```python
from build123d import *

# Parameters (mm, degrees)
BOSS_EXTRUDE7_DEPTH  = 3
SKETCH7_R            = 3.674588618
BOSS_EXTRUDE8_DEPTH  = 3.5
SKETCH8_R            = 3.674588618
BOSS_EXTRUDE9_DEPTH  = 3.5
SKETCH9_R            = 3.674588618
BOSS_EXTRUDE10_DEPTH = 3
SKETCH10_R           = 3.674588618
BOSS_EXTRUDE11_DEPTH = 3
SKETCH11_R           = 4.731271099
BOSS_EXTRUDE12_DEPTH = 1
SKETCH12_R           = 3.75
BOSS_EXTRUDE13_DEPTH = 7
BOSS_EXTRUDE14_START = 1
SKETCH13_R           = 4.731271099
BOSS_EXTRUDE14_DEPTH = 1
BOSS_EXTRUDE15_START = 7
SKETCH14_R           = 3.75
BOSS_EXTRUDE15_DEPTH = 7
CHAMFER1_SIZE        = 0.5


with BuildPart() as part:
    # Sketch1 → Boss-Extrude7 (new body)
    with BuildSketch(Plane.XY):
        with BuildLine():
            Line((-7.464079644, 5.007711231), (7.464079644, 5.007711231))
            ThreePointArc((7.464079644, 5.007711231), (12.46407809, 0.007713678), (7.464080538, -4.992284768))
            Line((7.464080538, -4.992284768), (-7.464079644, -4.992286102))
            ThreePointArc((-7.464079644, -4.992286102), (-12.464078311, 0.007712565), (-7.464079644, 5.007711231))
        make_face()
    extrude(amount=-BOSS_EXTRUDE7_DEPTH)

    # Sketch7 → Boss-Extrude8 (add)
    with BuildSketch(Plane(origin=(0, 0, -3), x_dir=(-1, 0, 0), z_dir=(0, 0, -1))):
        with Locations(Location((7.464079644, 0.007712565, 0), (0, 0, 180))):
            Circle(SKETCH7_R)
    extrude(amount=BOSS_EXTRUDE8_DEPTH)

    # Sketch8 → Boss-Extrude9 (add)
    with BuildSketch(Plane.XY):
        with Locations((7.464079644, 0.007712565)):
            Circle(SKETCH8_R)
    extrude(amount=BOSS_EXTRUDE9_DEPTH)

    # Sketch9 → Boss-Extrude10 (add)
    # profile 1 of 2: a face of its own
    with BuildSketch(Plane(origin=(0, 0, -6.5), x_dir=(-1, 0, 0), z_dir=(0, 0, -1))):
        with BuildLine():
            Line((7.458914982, 5.007708564), (-0.003874001, 5.003854283))
            ThreePointArc((-0.003874001, 5.003854283), (-5.003216645, -0.001949753), (0.003880454, -4.999997327))
            Line((0.003880454, -4.999997327), (7.464079644, -4.992284768))
            ThreePointArc((7.464079644, -4.992284768), (12.464077644, 0.007713232), (7.464079644, 5.007711231))
            Line((7.464079644, 5.007711231), (7.458914982, 5.007708564))
        make_face()
        with Locations(Location((7.464079644, 0.007712565, 0), (0, 0, 180))):
            Circle(SKETCH9_R, mode=Mode.SUBTRACT)
    # profile 2 of 2: a face of its own
    with BuildSketch(Plane(origin=(0, 0, -6.5), x_dir=(-1, 0, 0), z_dir=(0, 0, -1))):
        with Locations(Location((7.464079644, 0.007712565, 0), (0, 0, 180))):
            Circle(SKETCH9_R)
    extrude(amount=BOSS_EXTRUDE10_DEPTH)

    # Sketch10 → Boss-Extrude11 (add)
    # profile 1 of 2: a face of its own
    with BuildSketch(Plane.XY.offset(3.5)):
        with BuildLine():
            ThreePointArc((-0.003873651, 5.003854283), (-5.003216178, -0.00216555), (0.004312288, -4.999996973))
            Line((0.004312288, -4.999996973), (7.3891908, -4.991725236))
            ThreePointArc((7.3891908, -4.991725236), (12.463938092, -0.029732908), (7.464079644, 5.007711231))
            Line((7.464079644, 5.007711231), (7.458914981, 5.007708564))
            Line((7.458914981, 5.007708564), (-0.003873651, 5.003854283))
        make_face()
        with Locations((7.464079644, 0.007712565)):
            Circle(SKETCH10_R, mode=Mode.SUBTRACT)
    # profile 2 of 2: a face of its own
    with BuildSketch(Plane.XY.offset(3.5)):
        with Locations((7.464079644, 0.007712565)):
            Circle(SKETCH10_R)
    extrude(amount=BOSS_EXTRUDE11_DEPTH)

    # Sketch11 → Boss-Extrude12 (add)
    with BuildSketch(Plane.XY.offset(6.5)):
        with Locations((1e-09, 0.015425152)):
            Circle(SKETCH11_R)
    extrude(amount=BOSS_EXTRUDE12_DEPTH)

    # Sketch12 → Boss-Extrude13 (add)
    with BuildSketch(Plane.XY.offset(7.5)):
        with Locations((1e-09, 0.015425152)):
            Circle(SKETCH12_R)
    extrude(amount=BOSS_EXTRUDE13_DEPTH)

    # Sketch13 → Boss-Extrude14 (add)
    with BuildSketch(Plane(origin=(0, 0, -9.5), x_dir=(-1, 0, 0), z_dir=(0, 0, -1)).offset(BOSS_EXTRUDE14_START)):
        with Locations(Location((-1e-09, 0.015425152, 0), (0, 0, 180))):
            Circle(SKETCH13_R)
    extrude(amount=-BOSS_EXTRUDE14_DEPTH)

    # Sketch14 → Boss-Extrude15 (add)
    with BuildSketch(Plane(origin=(0, 0, -10.5), x_dir=(-1, 0, 0), z_dir=(0, 0, -1)).offset(BOSS_EXTRUDE15_START)):
        with Locations(Location((-1e-09, 0.015425152, 0), (0, 0, 180))):
            Circle(SKETCH14_R)
    extrude(amount=-BOSS_EXTRUDE15_DEPTH)

    # Chamfer1
    chamfer1_edges = [part.edges().sort_by_distance(p)[0] for p in [
        (-3.749999999, 0.015425152, 14.5),
        (-3.749999999, 0.015425152, -17.5),
    ]]
    chamfer(chamfer1_edges, length=CHAMFER1_SIZE)


solid = part.part
```
For this review, take the finished solid that the model builds, in its own axes (mm). A direction names the side the tool comes from. Round coordinates to 2 decimals unless told otherwise and drop trailing zeros. Order: outer loops, then holes, each group sorted by start corner. A loop starts at its lowest first (then second) coordinate and runs counter-clockwise, first axis right, second up. Notation, with made-up numbers: (51, 28) -> (108, 28) arc R11 cw to (108, 46) -> close; hole circle Ø9 at (-15, 34.5). An arc over 180 degrees is marked (long way). Use a Markdown table: item, result.
Item 1: Take a section at B-B (z = 6). State the section outline as (x, y) points, plus the area to 3 significant figures.
Resolved:
| item | result |
|---|---|
| outline | (0, -5) -> (7.39, -4.99) arc R5 ccw (long way) to (7.46, 5.01) -> (0, 5) arc R5 ccw to start |
| area | 153 mm² |
Item 2: Draft analysis for pull direction Z (two halves, no side actions). For faces 1 (the flat face through (-1, 4, 7.5)), 2 (the cylindrical face through (-11.135, -0.154, -4.726)), 3 (the flat face through (-7, 0, -9.5)), state which applies: +Z half, -Z half, draft (parallel to the pull), parting line (faces both ways), or undercut.
Resolved:
| item | result |
|---|---|
| face 1 | +Z half |
| face 2 | undercut |
| face 3 | -Z half |
Item 3: Machinability: for faces 4 (the cylindrical face through (-12.463, -0.102, -7.979)), 5 (the cylindrical face through (3.793, 0.169, 1.726)), 6 (the cylindrical face through (2.016, 3.177, 10.704)), which of the approach directions +Z, -Z, +X, -X, +Y, -Y give a long, thin tool a straight path to every point of the face, cutting with its end or side? Answer none if there is none.
Resolved:
| item | result |
|---|---|
| face 4 | +Z, -Z, -X |
| face 5 | none |
| face 6 | +Z |
Item 4: For line 1 along Z through (x, y) = (-1, 2); line 2 along Z through (x, y) = (1.75, -4.5); line 3 along Z through (x, y) = (11.75, 2), list the stretches that pass through material, from the lowest coordinate up. Write a range as [from, to].
Resolved:
| item | result |
|---|---|
| line 1 | z = [-17.5, -6.5], [-3, 0], [3.5, 14.5] |
| line 2 | z = [-9.5, -6.5], [-3, 0], [3.5, 6.5] |
| line 3 | z = [-3, 0], [3.5, 6.5] |
Item 5: For pin 1 (6 mm diameter, centred on x = 1, z = 8.5, fed in from +Y); pin 2 (4 mm diameter, centred on y = -4, z = 4, fed in from +X); pin 3 (1.5 mm diameter, centred on x = 3, z = -1, fed in from -Y), all flat-tipped, find the tip position at first contact; note any pin that passes through.
Resolved:
| item | result |
|---|---|
| pin 1 | stops at y = 5.01 |
| pin 2 | stops at x = 12.04 |
| pin 3 | stops at y = -4.99 |
Item 6: Take a section at D-D (x = 1.75). State how many separate pieces and enclosed holes the cut face has, plus the area to 3 significant figures.
Resolved:
| item | result |
|---|---|
| separate pieces | 3 |
| enclosed holes | 0 |
| area | 198 mm² |
Item 7: Take a section at A-A (x = -4.25). State the section outline as (y, z) points, plus the area to 3 significant figures.
Resolved:
| item | result |
|---|---|
| outline | (-5, -9.5) -> (-2.06, -9.5) -> (-2.06, -10.5) -> (2.09, -10.5) -> (2.09, -9.5) -> (5.01, -9.5) -> (5.01, -6.5) -> (1.79, -6.5) -> (1.79, -3) -> (5.01, -3) -> (5.01, 0) -> (-4.99, 0) -> (-4.99, -3) -> (-1.77, -3) -> (-1.77, -6.5) -> (-5, -6.5) -> close; (-2.64, 3.5) -> (2.64, 3.5) -> (2.64, 6.5) -> (2.09, 6.5) -> (2.09, 7.5) -> (-2.06, 7.5) -> (-2.06, 6.5) -> (-2.64, 6.5) -> close |
| area | 96.6 mm² |
Item 8: Take a section at C-C (x = 9). State the section outline as (y, z) points.
Resolved:
| item | result |
|---|---|
| outline | (-4.75, -3) -> (4.77, -3) -> (4.77, 0) -> (3.35, 0) -> (3.35, 3.5) -> (4.77, 3.5) -> (4.77, 6.5) -> (-4.75, 6.5) -> (-4.75, 3.5) -> (-3.33, 3.5) -> (-3.33, 0) -> (-4.75, 0) -> close |
